Check sheet for the drawn part. Datum: minimum x, y, z corner. Units: mm. A direction names the side the tool comes from. Round coordinates to 2 decimals unless told otherwise and drop trailing zeros. Loops run counter-clockwise (first coordinate to the right, second up) from the corner with the lowest first, then second, coordinate; pieces in that order, holes last.
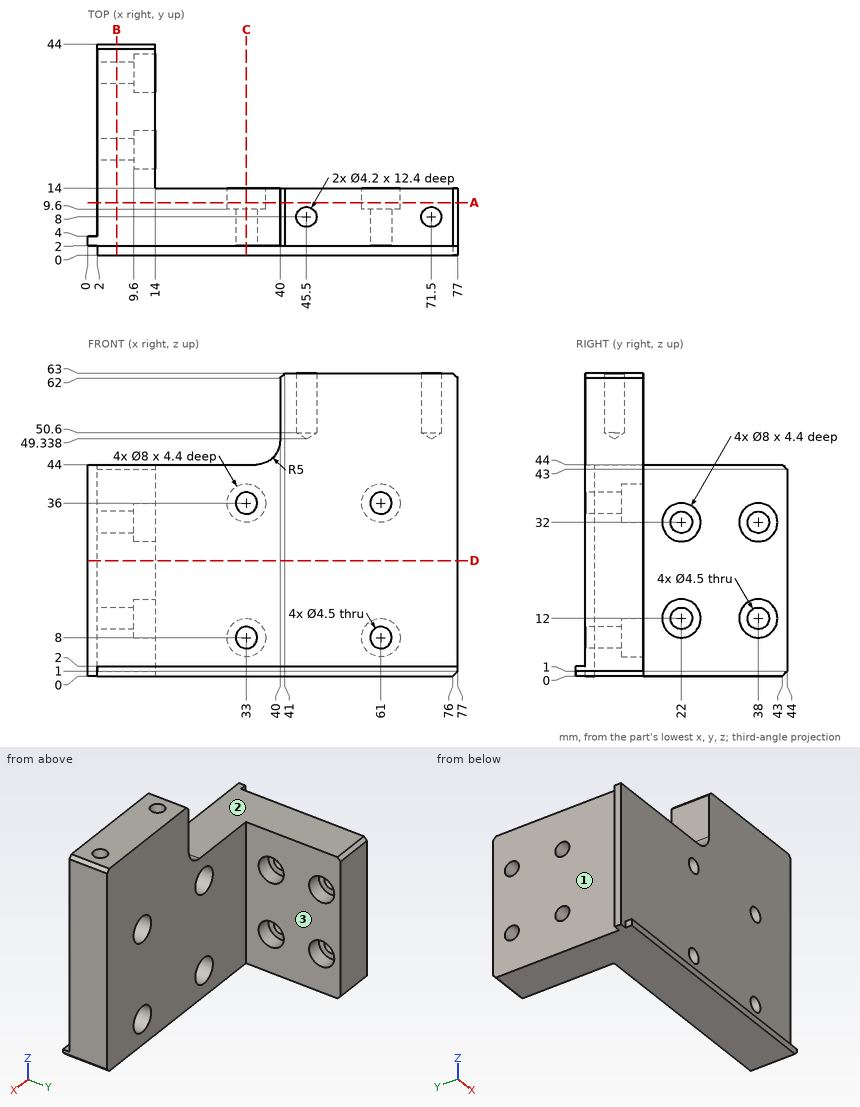
1. Section check C-C (x = 33). Enter the section's corners in (y, z).
2. Section check B-B (x = 6). Enter the section's corners in (y, z), then the cut area to 3 significant figures.
3. Gauge pin test, flat ends, axial feed: P1, Ø4, axis at x = 34, z = 34.5, coming from the +Y side; P2, Ø8, axis at x = 61, z = 14.5, coming from the -Y side; P3, Ø3, axis at x = 31.5, y = 7, coming from the +Z side. Record the tip position at first contact, or that the pin passes through.
4. Tool access check on the marked faces 1, 2 and 3. Record the directions out of +Z, -Z, +X, -X, +Y, -Y that give a thin tool (end or side, any length) a straight path to the whole face; none if there is none.
5. Section check A-A (y = 11). Enter the section's corners in (x, z), then the cut area to 3 significant figures.
6. Scan lines: L1, parallel to Y at x = 5.75, z = 32; L2, parallel to X at y = 8, z = 56; L3, parallel to X at y = 13.5, z = 9. Record each from-to range of solid material in increasing order.
7. Section check D-D (z = 24). Enter the section's corners in (x, y), then the cut area to 3 significant figures.
Taken from the geometry:
1. outline: (0, 0) - (14, 0) - (14, 4) - (9.6, 4) - (9.6, 5.75) - (2, 5.75) - (2, 2) - (0, 2) - close; (2, 10.25) - (9.6, 10.25) - (9.6, 12) - (14, 12) - (14, 32) - (9.6, 32) - (9.6, 33.75) - (2, 33.75) - close; (2, 38.25) - (9.6, 38.25) - (9.6, 40) - (14, 40) - (14, 44) - (2, 44) - close
2. outline: (0, 0) - (43, 0) - (44, 1) - (44, 43) - (43, 44) - (2, 44) - (2, 2) - (0, 2) - close; hole circle Ø4.5 at (22, 12); hole circle Ø4.5 at (22, 32); hole circle Ø4.5 at (38, 12); hole circle Ø4.5 at (38, 32)
2. area: 1,790 mm2
3. P1: stops at y = 9.6
3. P2: stops at y = 2
3. P3: stops at z = 44
4. face 1: +Z, -Z, -X, +Y
4. face 2: +Z, -X, +Y, -Y
4. face 3: +Z, -Z, +X, +Y
5. outline: (2, 0) - (76, 0) - (77, 1) - (77, 62) - (76, 63) - (41, 63) - (40, 62) - (40, 49) arc R5 cw to (35, 44) - (2, 44) - close; hole circle Ø8 at (33, 8); hole circle Ø8 at (33, 36); hole circle Ø8 at (61, 8); hole circle Ø8 at (61, 36)
5. area: 3,810 mm2
6. L1: y = 2 to 19.75, 24.25 to 35.75, 40.25 to 44
6. L2: x = 40 to 43.4, 47.6 to 69.4, 73.6 to 77
6. L3: x = 2 to 29.13, 36.87 to 57.13, 64.87 to 77
7. outline: (0, 2) - (77, 2) - (77, 14) - (14, 14) - (14, 44) - (2, 44) - (2, 4) - (0, 4) - close
7. area: 1,260 mm2
